Drawing for the job (mm, zero at the part's lowest x, y, z). A direction names the side the tool comes from. Coordinates: 2 decimals unless noted, no trailing zeros. Write each loop counter-clockwise with the first axis right and the second up, starting at its lowest first coordinate (ties: lowest second). Pieces come first, ordered by that corner, then holes. Notation, with made-up numbers: (45.25, 12) - (58.25, 12) arc R17 cw to (58.25, 21) - close; hole circle Ø5 at (65, 61). An arc over 180 degrees is marked (long way). Write each question's results on one line, items separated by ' | '.
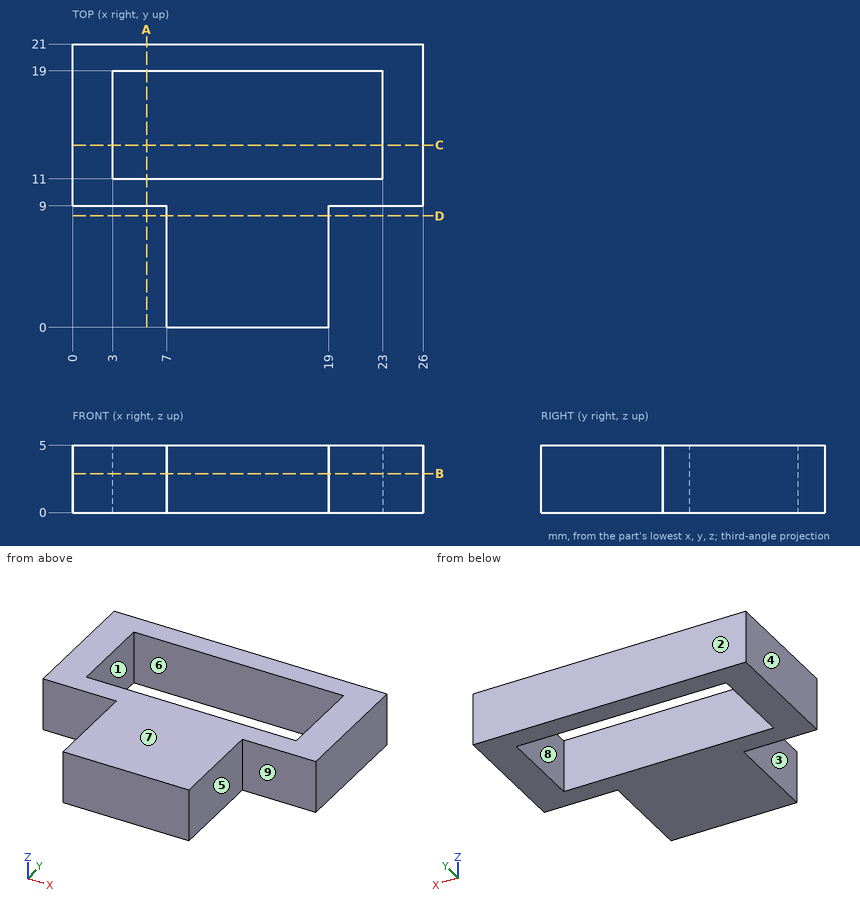
(1) Flat gauge pins, fed straight in: P1, Ø1.5, axis at x = 15, y = 17.5, coming from the -Z side; P2, Ø2.5, axis at x = 22.5, z = 2.5, coming from the -Y side. Where does each tip first touch, or does it go through?
Return value:
P1: passes through | P2: stops at y = 9
(2) 3-axis set-ups, long thin cutter, end or side, ignore diameter. For the marked faces 1, 2, 3, 4 and 5: which of +Z, -Z, +X, -X, +Y, -Y reach the whole face in a straight line?
Return value:
face 1: +Z, -Z | face 2: +Z, -Z, +X, -X, +Y | face 3: +Z, -Z, -X, -Y | face 4: +Z, -Z, -X, +Y, -Y | face 5: +Z, -Z, +X, -Y
(3) Saw through at B-B on z = 2.9. Write the cut outline in (x, y), then the cut area to 3 significant figures.
Return value:
outline: (0, 9) - (7, 9) - (7, 0) - (19, 0) - (19, 9) - (26, 9) - (26, 21) - (0, 21) - close; hole (3, 11) - (23, 11) - (23, 19) - (3, 19) - close | area: 260 mm^2
(4) Saw through at D-D on y = 8.25. Write the cut outline in (x, z), then the cut area to 3 significant figures.
Return value:
outline: (7, 0) - (19, 0) - (19, 5) - (7, 5) - close | area: 60.0 mm^2
(5) Saw through at C-C on y = 13.5. Write the cut outline in (x, z).
Return value:
outline: (0, 0) - (3, 0) - (3, 5) - (0, 5) - close; (23, 0) - (26, 0) - (26, 5) - (23, 5) - close
(6) Wall check: line 1 (Y direction, x = 19.5, z = 1.5); line 2 (X direction, y = 13, z = 1.2); line 3 (Y direction, x = 15.5, z = 0.3). Give the ranges that are in metal, low to high. Write a range as from..to.
Return value:
line 1: y = 9..11, 19..21 | line 2: x = 0..3, 23..26 | line 3: y = 0..11, 19..21
(7) Two-plate mould, pull along Y, no slides. Class the marked faces 6, 7, 8 and 9: released by +Y, released by -Y, zero draft, split by the parting line, or undercut.
Return value:
face 6: undercut | face 7: zero draft | face 8: undercut | face 9: released by -Y
(8) Saw through at A-A on x = 5.5. Write the cut outline in (y, z).
Return value:
outline: (9, 0) - (11, 0) - (11, 5) - (9, 5) - close; (19, 0) - (21, 0) - (21, 5) - (19, 5) - close
